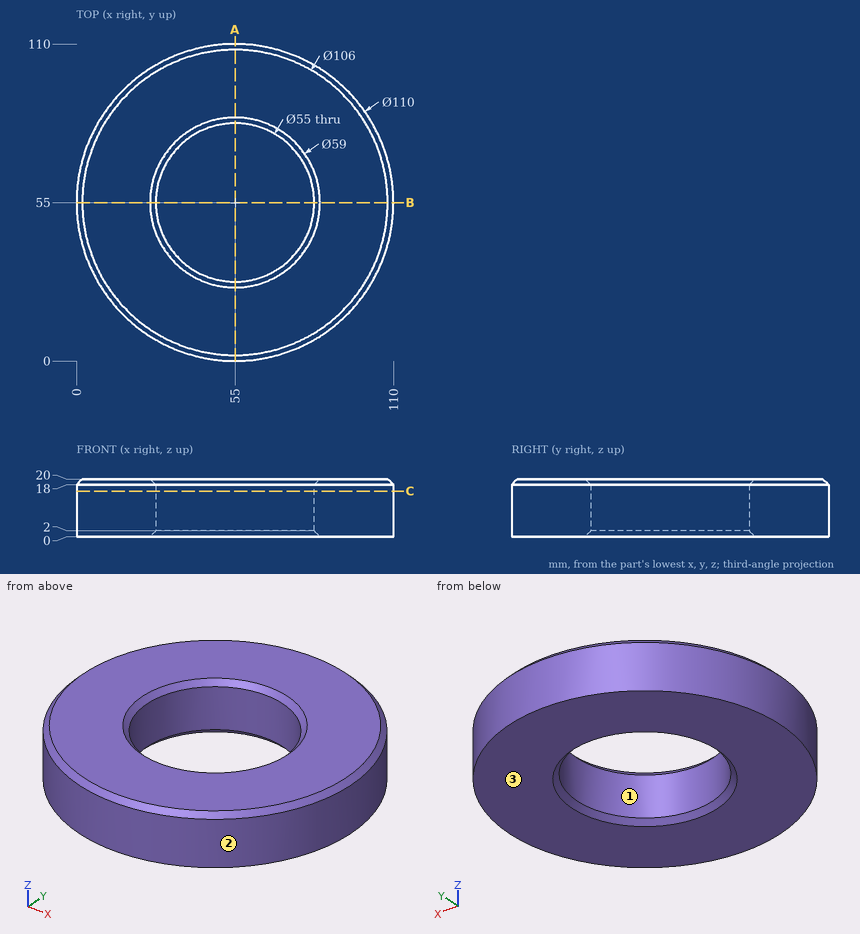
The figure shows three views and two pictorial views of one solid part (mm, origin at its lowest corner). Answer the questions. Give positions to 0.01 mm unless a question says otherwise; leave off trailing zeros. Loops run counter-clockwise (first coordinate to the right, second up) from the corner with the lowest first, then second, coordinate; pieces in that order, holes last. Notation, with made-up numbers: (-17.75, 24) -> (10.25, 24) arc R20 cw to (10.25, 55) -> close; hole circle Ø1 at (64.5, 47.25). An arc over 180 degrees is marked (long way). Use a Markdown table: item, result. Add a question column.
1. Flat-ended cylindrical pins translate along their axes: pin 1 Ø8 at (y, z) = (26.5, 3.5) entering from -X; pin 2 Ø2 at (y, z) = (27.5, 14.5) entering from -X; pin 3 Ø12 at (y, z) = (23, 7) entering from -X. Find the tip coordinate at first contact, or state that the pin passes through.
2. Find the intervals of material crossed by probe 1 along Y at (x, z) = (55, 6.5); probe 2 along Y at (x, z) = (47.5, 8); probe 3 along X at (y, z) = (51, 15.75), in increasing order.
3. Section A-A on x = 55 is taken. Determine the outline of the cut face in (y, z).
4. Determine the mould class of the marked faces 1, 2 and 3 for opening direction Y: released by +Y, released by -Y, zero draft, split by the parting line, or undercut.
5. Section C-C on z = 15.75 is taken. Determine the outline of the cut face in (x, y).
Results below:
| question | item | result |
|---|---|---|
| 1 | pin 1 | stops at x = 5.76 |
| 1 | pin 2 | stops at x = 6.81 |
| 1 | pin 3 | stops at x = 6.53 |
| 2 | probe 1 | y = 0 to 27.5, 82.5 to 110 |
| 2 | probe 2 | y = 0.51 to 28.54, 81.46 to 109.49 |
| 2 | probe 3 | x = 0.15 to 27.79, 82.21 to 109.85 |
| 3 | outline | (0, 0) -> (25.5, 0) -> (27.5, 2) -> (27.5, 18) -> (25.5, 20) -> (2, 20) -> (0, 18) -> close; (82.5, 2) -> (84.5, 0) -> (110, 0) -> (110, 18) -> (108, 20) -> (84.5, 20) -> (82.5, 18) -> close |
| 4 | face 1 | undercut |
| 4 | face 2 | split by the parting line |
| 4 | face 3 | zero draft |
| 5 | outline | circle Ø110 at (55, 55); hole circle Ø55 at (55, 55) |
